```python
from build123d import *

# Parameters (mm, degrees)
EXTRUDE_1_DEPTH              = 15
HOLE_WIZARD_M5_1_D           = 5.5
HOLE_WIZARD_M5_1_CBORE_D     = 10
HOLE_WIZARD_M5_1_CBORE_DEPTH = 42
SKETCH_4_W                   = 32
SKETCH_4_H                   = 27
CUT_EXTRUDE_2_DEPTH          = 60.699246397
CUT_EXTRUDE_3_DEPTH          = 49.476798739
FILLET_1_R                   = 2
FILLET_2_R                   = 3
CHAMFER_1_SIZE               = 0.5


with BuildPart() as part:
    # 草圖1 → 伸長1 (new, symmetric)
    with BuildSketch(Plane.XY):
        with BuildLine():
            Line((-30, 0), (30, 0))
            Line((30, 0), (30, 12))
            ThreePointArc((30, 12), (0, 42), (-30, 12))
            Line((-30, 12), (-30, 0))
        make_face()
    extrude(amount=EXTRUDE_1_DEPTH, both=True)

    # M5 六角承窩頭蓋螺釘的柱孔1 (through all)
    with Locations(Plane(origin=(0, 50, 0), x_dir=(1, 0, 0), z_dir=(0, 1, 0))):
        with Locations((-24, 0), (24, 0)):
            CounterBoreHole(HOLE_WIZARD_M5_1_D / 2, HOLE_WIZARD_M5_1_CBORE_D / 2, HOLE_WIZARD_M5_1_CBORE_DEPTH)

    # 草圖4 → 伸長2 (cut, through all)
    with BuildSketch(Plane.XY.offset(15)):
        with Locations((0, 20.5)):
            Rectangle(SKETCH_4_W, SKETCH_4_H)
    extrude(amount=-CUT_EXTRUDE_2_DEPTH, mode=Mode.SUBTRACT)

    # 草圖5 → 伸長3 (cut, through all)
    with BuildSketch(Plane(origin=(0, 7, 0), x_dir=(1, 0, 0), z_dir=(0, 1, 0))):
        Polygon((-16, 15), (-16, 5), (-7.25, 5), (-7.25, -8), (7.25, -8), (7.25, 5), (16, 5), (16, 15), align=None)
    extrude(amount=-CUT_EXTRUDE_3_DEPTH, mode=Mode.SUBTRACT)

    # 圓角1
    fillet_1_edges = [part.edges().sort_by_distance(p)[0] for p in [
        (-16, 34, 0),
        (16, 34, 0),
        (16, 7, 5),
        (-16, 7, 5),
    ]]
    fillet(fillet_1_edges, radius=FILLET_1_R)

    # 圓角2
    fillet_2_edges = [part.edges().sort_by_distance(p)[0] for p in [
        (30, 6, 15),
        (0, 42, 15),
        (-30, 6, 15),
        (0, 42, -15),
        (30, 6, -15),
        (-30, 6, -15),
    ]]
    fillet(fillet_2_edges, radius=FILLET_2_R)

    # 導角1
    chamfer_1_edges = [part.edges().sort_by_distance(p)[0] for p in [
        (16, 16, -15),
        (16, 20.5, 15),
        (0, 7, 15),
        (-16, 20.5, 15),
        (-16, 16, -15),
        (0, 34, 15),
        (0, 34, -15),
        (15.414213562, 7.585786438, 15),
        (-15.414213562, 7.585786438, 15),
        (-15.414213562, 33.414213562, 15),
        (-15.414213562, 33.414213562, -15),
        (15.414213562, 33.414213562, 15),
        (15.414213562, 33.414213562, -15),
    ]]
    chamfer(chamfer_1_edges, length=CHAMFER_1_SIZE)


solid = part.part
```
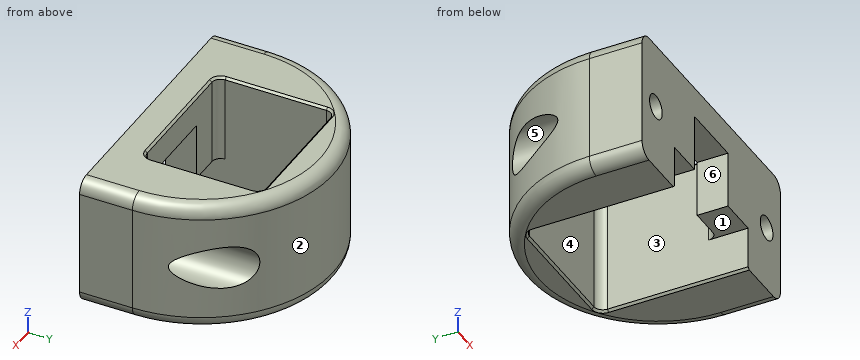
Here's how the part is built. I have some questions about the finished solid (model axes, mm). Face numbers are marked on the shaded views. A direction names the side the tool comes from. Round coordinates to 2 decimals unless told otherwise and drop trailing zeros. Write each loop counter-clockwise with the first axis right and the second up, starting at its lowest first coordinate (ties: lowest second). Pieces come first, ordered by that corner, then holes. Notation, with made-up numbers: M 50,-6.5 L 83,-6.5 A8 cw 83,8.5 Z; hole C 28,-29 d4. An arc over 180 degrees is marked long. Answer as CSV lines item,"result". Start each with the question number.
1. I'm going to push flat-ended pins straight in: pin 1 Ø4.5 at (x, y) = (11.5, 3) entering from -Z; pin 2 Ø3.5 at (x, y) = (1.5, 4) entering from -Z; pin 3 Ø16 at (x, z) = (24, 0) entering from +Y; pin 4 Ø4.5 at (x, z) = (24, 0) entering from +Y. Where does each tip first touch, or does it pass through?
2. Suppose I cut it at A-A on z = 9.5. Write out the boundary of the cut face in (x, y), then the cut area to 3 significant figures.
3. Thinking about a two-plate mould opening in Y: for the marked faces 1, 2 and 3, which applies, released by +Y, released by -Y, zero draft, split by the parting line, or undercut?
4. On a 3-axis mill with a long thin cutter (end or side, diameter ignored), from which of +Z, -Z, +X, -X, +Y, -Y can I reach the whole of each face in a straight line? I mean the marked faces 4, 5 and 6. Say none if no direction works.
5. Suppose I cut it at B-B on z = 3.5. Write out the boundary of the cut face in (x, y).
6. I need wall thicknesses on probe 1 along Z at (x, y) = (-24, 14.5); probe 2 along Z at (x, y) = (-24, 5); probe 3 along X at (y, z) = (16.5, -3). Which ranges of each line are inside material? Lowest first, please.
Check result:
1,pin 1,"stops at z = -5"
1,pin 2,"stops at z = 8"
1,pin 3,"stops at y = 37.38"
1,pin 4,"passes through"
2,outline,"M -30,0 L 30,0 L 30,12 A30 ccw -30,12 Z; hole M -16,9 A2 ccw -14,7 L 14,7 A2 ccw 16,9 L 16,32 A2 ccw 14,34 L -14,34 A2 ccw -16,32 Z"
2,area,"1,270 mm2"
3,face 1,"zero draft"
3,face 2,"released by +Y"
3,face 3,"undercut"
4,face 4,"+Z, -Z"
4,face 5,"+Y"
4,face 6,"-Z, -Y"
5,outline,"M -30,0 L -7.25,0 L -7.25,7 L -14,7 A2 cw -16,9 L -16,32 A2 cw -14,34 L 14,34 A2 cw 16,32 L 16,9 A2 cw 14,7 L 7.25,7 L 7.25,0 L 30,0 L 30,12 A30 ccw 27.57,23.83 L 27.57,8 L 20.43,8 L 20.43,33.97 A30 ccw -20.43,33.97 L -20.43,8 L -27.57,8 L -27.57,23.83 A30 ccw -30,12 Z"
6,probe 1,"z = -15 to -5, 5 to 15"
6,probe 2,"z = -15 to -2.75, 2.75 to 15"
6,probe 3,"x = -29.66 to -28, -20 to -16, 16 to 20, 28 to 29.66"
